The listing builds one solid part. Answer for the finished solid, in the listing's coordinates (mm). Coordinates: 2 decimals unless noted, no trailing zeros. Write each loop counter-clockwise with the first axis right and the second up, starting at its lowest first coordinate (ties: lowest second). Pieces come first, ordered by that corner, then holes. Notation, with made-up numbers: M 5,65.25 L 13,65.25 A17 ccw 13,87.25 Z; hole C 66.5,-37.5 d5. An arc over 180 degrees is marked long. Put each result on its own line as item: value. Start each with the question number.
```python
from build123d import *

# Parameters (mm, degrees)
BOSS_EXTRUDE1_DEPTH   = 10
CHAMFER1_SIZE         = 25
FILLET1_R             = 20
F_26_DIAMETER_HOLE1_D = 26


with BuildPart() as part:
    # Sketch1 → Boss-Extrude1 (new, symmetric)
    with BuildSketch(Plane.XY):
        Polygon((0, 0), (0, 695), (90, 695), (90, 654), (600, 654), (600, 294), (290, 294), (140, 0), align=None)
    extrude(amount=BOSS_EXTRUDE1_DEPTH, both=True)

    # Chamfer1
    chamfer1_edges = [part.edges().sort_by_distance(p)[0] for p in [
        (0, 0, 0),
        (0, 695, 0),
    ]]
    chamfer(chamfer1_edges, length=CHAMFER1_SIZE)

    # Fillet1
    fillet1_edges = [part.edges().sort_by_distance(p)[0] for p in [
        (90, 654, 0),
        (600, 654, 0),
        (600, 294, 0),
        (290, 294, 0),
    ]]
    fillet(fillet1_edges, radius=FILLET1_R)

    # Ø26 Diameter Hole1 (through all)
    with Locations(Plane.XY.offset(10)):
        with Locations((181.5, 621), (476.5, 621), (476.5, 381), (181.5, 381)):
            Hole(F_26_DIAMETER_HOLE1_D / 2)


solid = part.part
```
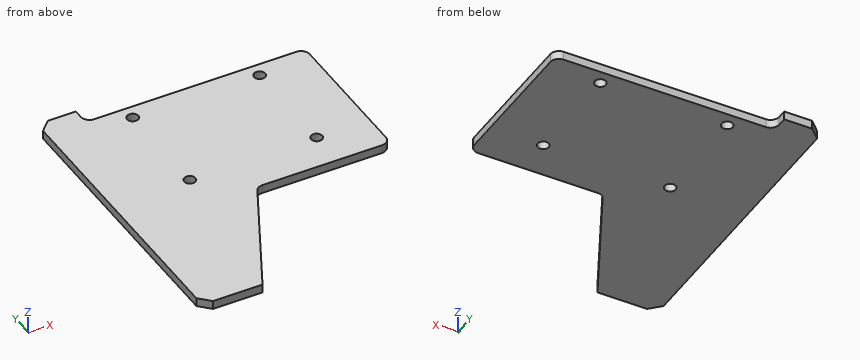
1) A cutting plane is placed at D-D on x = 252. Write down the section's boundary in (y, z), then the cut area to 3 significant figures.
2) Given pin 1 Ø1.5 at (y, z) = (150, -2) entering from +X; pin 2 Ø1.5 at (x, z) = (197.5, 3) entering from +Y; pin 3 Ø23.5 at (x, y) = (476.5, 621) entering from +Z, each flat-ended and moving along its own axis, determine where each tip first touches the part or whether it passes through.
3) A cutting plane is placed at C-C on y = 381. Write down the section's boundary in (x, z).
4) A cutting plane is placed at B-B on z = 4.75. Write down the section's boundary in (x, y).
5) A cutting plane is placed at A-A on x = 181.5. Write down the section's boundary in (y, z).
6) Straight lines are drawn through the part: probe 1 along Y at (x, z) = (476.5, -4.5); probe 2 along X at (y, z) = (621, -5); probe 3 along Y at (x, z) = (181.5, 4.25). For each, find the intervals that lie inside material, in ascending order.
Answers follow:
1. outline: M 219.52,-10 L 654,-10 L 654,10 L 219.52,10 Z
1. area: 8,690 mm²
2. pin 1: stops at x = 216.91
2. pin 2: stops at y = 654
2. pin 3: passes through
3. outline: M 0,-10 L 168.5,-10 L 168.5,10 L 0,10 Z; M 194.5,-10 L 463.5,-10 L 463.5,10 L 194.5,10 Z; M 489.5,-10 L 600,-10 L 600,10 L 489.5,10 Z
4. outline: M 0,25 L 25,0 L 140,0 L 284.43,283.09 A20 cw 302.25,294 L 580,294 A20 ccw 600,314 L 600,634 A20 ccw 580,654 L 110,654 A20 cw 90,674 L 90,695 L 25,695 L 0,670 Z; hole C 181.5,381 d26; hole C 181.5,621 d26; hole C 476.5,381 d26; hole C 476.5,621 d26
5. outline: M 81.34,-10 L 368,-10 L 368,10 L 81.34,10 Z; M 394,-10 L 608,-10 L 608,10 L 394,10 Z; M 634,-10 L 654,-10 L 654,10 L 634,10 Z
6. probe 1: y = 294 to 368, 394 to 608, 634 to 654
6. probe 2: x = 0 to 168.5, 194.5 to 463.5, 489.5 to 600
6. probe 3: y = 81.34 to 368, 394 to 608, 634 to 654
